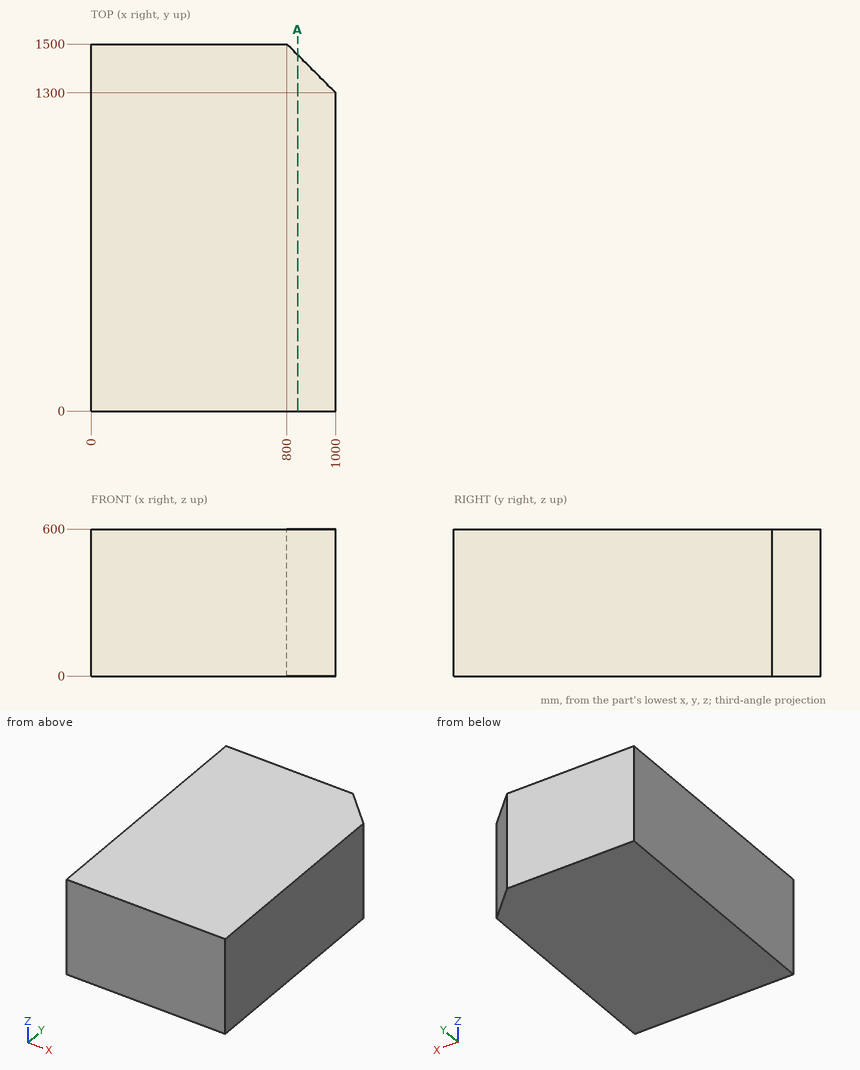
Could you check a few things on this drawing? It's one solid part, dimensions in mm from its lowest x, y, z. Give positions to 0.01 mm unless a question says otherwise; leave off trailing zeros. Order: outer loops, then holes, each group sorted by start corner. A loop starts at its lowest first (then second) coordinate and runs counter-clockwise, first axis right, second up. Notation, with made-up numbers: (19, -13) - (46, -13) arc R20 cw to (46, -4) - close; hole circle Ø4 at (82, -11). An arc over 180 degrees is marked (long way). Return JSON: item names as keys, results as strings. Group by question number.
Q1. Will this pin go through, and if not, where does the flat tip stop? pin 1 Ø2 at (x, z) = (897, 537.5) entering from -Y.
Q2. Suppose I cut it at A-A, the plane x = 843.5. Please give me the cut outline in (y, z), and give its area (3 significant figures).
Q3. Please list where these lines run through material, in increasing order: line 1 along Y through (x, z) = (941, 542); line 2 along X through (y, z) = (1429.5, 488); line 3 along Y through (x, z) = (813, 198). Write a range as [from, to].
Resolved:
{
 "1": {"pin 1": "stops at y = 0"},
 "2": {"outline": "(0, 0) - (1456.5, 0) - (1456.5, 600) - (0, 600) - close", "area": "874,000 mm2"},
 "3": {"line 1": "y = [0, 1359]", "line 2": "x = [0, 870.5]", "line 3": "y = [0, 1487]"}
}
